from build123d import *

# Parameters (mm, degrees)
SWEEP1_PROFILE_R    = 14
SHELL1_T            = -2
BOSS_EXTRUDE1_START = -6
SKETCH6_R           = 20
SKETCH6_R_2         = 12
SKETCH6_R_3         = 1.5
BOSS_EXTRUDE1_DEPTH = 3


with BuildPart() as part:
    # Sweep1: sweep along a path in Sketch1
    with BuildLine(Plane.XY) as sweep1_path:
        Line((0, 0), (0, -70))
        ThreePointArc((0, -70), (-8.786796564, -91.213203436), (-30, -100))
        Line((-30, -100), (-102, -100))
    # Sweep1 profile (on start of the path) → Sweep1 (sweep)
    with BuildSketch(Plane(origin=(0, 0, 0), x_dir=(-1, 0, 0), z_dir=(0, -1, 0))):
        Circle(SWEEP1_PROFILE_R)
    sweep(path=sweep1_path.line)

    # Shell1
    shell1_openings = [part.faces().sort_by_distance(p)[0] for p in [
        (-102, -100, 0),
        (0, 0, 0),
    ]]
    offset(amount=SHELL1_T, openings=shell1_openings, kind=Kind.INTERSECTION)

    # Sketch6 → Boss-Extrude1 (add)
    with BuildSketch(Plane.ZY.offset(102).offset(BOSS_EXTRUDE1_START)):
        with Locations((0, -100)):
            Circle(SKETCH6_R)
        with Locations(Location((0, -100, 0), (0, 0, 270))):
            Circle(SKETCH6_R_2, mode=Mode.SUBTRACT)
        with Locations((0, -82)):
            Circle(SKETCH6_R_3, mode=Mode.SUBTRACT)
        with Locations((18, -100)):
            Circle(SKETCH6_R_3, mode=Mode.SUBTRACT)
        with Locations((0, -118)):
            Circle(SKETCH6_R_3, mode=Mode.SUBTRACT)
        with Locations((-18, -100)):
            Circle(SKETCH6_R_3, mode=Mode.SUBTRACT)
    extrude(amount=-BOSS_EXTRUDE1_DEPTH)


solid = part.part
Input: part model. Units: mm. Frame: model coordinates. A direction names the side the tool comes from. Coordinates: 2 decimals unless noted, no trailing zeros. Loops run counter-clockwise (first coordinate to the right, second up) from the corner with the lowest first, then second, coordinate; pieces in that order, holes last.
(1) Section B-B on y = -118. Return the cut outline in (x, z), then the cut area to 3 significant figures.
(2) Set-up query: faces 1 (the face through (-94.521, -116.513, -0.195)), 2 (the face through (-66.5, -111.99, -0.53)), 3 (the face through (11.99, -35.49, -0.53)), 4 (the face through (-93, -106, -13)). Return all of +Z, -Z, +X, -X, +Y, -Y with unobstructed straight access to the full face (end or side cutting, diameter ignored); none if empty.
(3) Section D-D on x = -83.5. Return the cut outline in (y, z), then the cut area to 3 significant figures.
(4) Section A-A on z = 0. Count the separate pieces of the cut face and the enclosed holes in it, then the cut area to 3 significant figures.
(5) First-contact query: pin 1 Ø3.5 at (y, z) = (-100, -18) entering from -X; pin 2 Ø5 at (y, z) = (-118, 0) entering from +X; pin 3 Ø6 at (x, y) = (-34.5, -106.5) entering from +Z; pin 4 Ø12 at (y, z) = (-106.5, 2.5) entering from -X. Flat tips, straight axial feed; report the tip coordinate or a pass-through.
(6) Pull-direction query (Y, two-part tool) for faces 5 (the face through (-94.521, -98.513, -18.195)), 6 (the face through (10.4, 0, 6.3)), 7 (the face through (-12.932, -35.49, 5.362)); classes: released by +Y, released by -Y, zero draft, split by the parting line, or undercut.
(7) Section C-C on z = -18. Return the cut outline in (x, y), then the cut area to 3 significant figures.
(8) Material intervals for probe 1 along Y at (x, z) = (-93.8, 0); probe 2 along Y at (x, z) = (-48.5, 0); probe 3 along Z at (x, y) = (-44, -100), sorted ascending.
Data:
1. outline: (-96, -8.72) - (-93, -8.72) - (-93, -1.5) - (-96, -1.5) - close; (-96, 1.5) - (-93, 1.5) - (-93, 8.72) - (-96, 8.72) - close
1. area: 43.3 mm2
2. face 1: +X, -X
2. face 2: -X
2. face 3: +Y
2. face 4: none
3. outline: circle Ø28 at (-100, 0); hole circle Ø24 at (-100, 0)
3. area: 163 mm2
4. separate pieces: 4
4. enclosed holes: 0
4. area: 774 mm2
5. pin 1: stops at x = -96
5. pin 2: stops at x = -93
5. pin 3: stops at z = 13.56
5. pin 4: stops at x = -102
6. face 5: undercut
6. face 6: released by +Y
6. face 7: zero draft
7. outline: (-96, -108.72) - (-93, -108.72) - (-93, -101.5) - (-96, -101.5) - close; (-96, -98.5) - (-93, -98.5) - (-93, -91.28) - (-96, -91.28) - close
7. area: 43.3 mm2
8. probe 1: y = -120 to -119.5, -116.5 to -112, -88 to -83.5, -80.5 to -80
8. probe 2: y = -114 to -112, -88 to -86
8. probe 3: z = -14 to -12, 12 to 14
